Read the model definition and answer for the solid it produces. Units are mm, in the model's axes. A direction names the side the tool comes from. Coordinates: 2 decimals unless noted, no trailing zeros. Order: outer loops, then holes, each group sorted by start corner. A loop starts at its lowest first (then second) coordinate and runs counter-clockwise, first axis right, second up. Notation, with made-up numbers: (17, 84.5) - (22, 84.5) arc R19 cw to (22, 115.5) - close; hole circle Ø10 at (39, -32). An arc over 180 degrees is marked (long way). Write item = value, one per line.
from build123d import *

# Parameters (mm, degrees)
BASE_BLOCK_DEPTH             = 60
SADDLE_ARCH_DEPTH            = 60
BEARING_SEAT_CUT_FRONT_DEPTH = 10
BEARING_START                = -10
BEARING_SEAT_CUT_REAR_DEPTH  = 10
OIL_HOLE_SKETCH_R            = 8
OIL_HOLE_8_DEPTH             = 100
LOCATING_SLOTS_SKETCH_W      = 8
LOCATING_SLOTS_SKETCH_H      = 16
LOCATING_SLOTS_DEPTH         = 9


with BuildPart() as part:
    # Base Block Profile → Base Block (new body)
    with BuildSketch(Plane.XY):
        Polygon((0, 0), (53, 0), (53, 12), (70, 12), (70, 32), (44.5, 32), (44.508364197, 12), (8.257120322, 12), (8.257120322, 32), (-17, 32), (-17, 12), (0, 12), align=None)
    extrude(amount=-BASE_BLOCK_DEPTH)

    # Saddle Arch Profile → Saddle Arch (add)
    with BuildSketch(Plane.XY):
        with BuildLine():
            Line((1.378560161, 32), (8.257120322, 32))
            Line((8.257120322, 32), (8.378560161, 32))
            ThreePointArc((8.378560161, 32), (26.378560161, 50), (44.378560161, 32))
            Line((44.378560161, 32), (44.5, 32))
            Line((44.5, 32), (51.378560161, 32))
            ThreePointArc((51.378560161, 32), (26.378560161, 57), (1.378560161, 32))
        make_face()
    extrude(amount=-SADDLE_ARCH_DEPTH)

    # Bearing Seat Front Profile → Bearing Seat Cut Front (cut)
    with BuildSketch(Plane.XY):
        with BuildLine():
            Line((1.378560161, 32), (8.257120322, 32))
            Line((8.257120322, 32), (8.378560161, 32))
            ThreePointArc((8.378560161, 32), (26.378560161, 50), (44.378560161, 32))
            Line((44.378560161, 32), (44.5, 32))
            Line((44.5, 32), (51.378560161, 32))
            ThreePointArc((51.378560161, 32), (26.378560161, 57), (1.378560161, 32))
        make_face()
    extrude(amount=-BEARING_SEAT_CUT_FRONT_DEPTH, mode=Mode.SUBTRACT)

    # Bearing Seat Rear Profile → Bearing Seat Cut Rear (cut)
    with BuildSketch(Plane(origin=(0, 0, -60), x_dir=(-1, 0, 0), z_dir=(0, 0, -1)).offset(BEARING_START)):
        with BuildLine():
            Line((-51.378560161, 32), (-44.378560161, 32))
            ThreePointArc((-44.378560161, 32), (-26.378560161, 50), (-8.378560161, 32))
            Line((-8.378560161, 32), (-1.378560161, 32))
            ThreePointArc((-1.378560161, 32), (-26.378560161, 57), (-51.378560161, 32))
        make_face()
    extrude(amount=BEARING_SEAT_CUT_REAR_DEPTH, mode=Mode.SUBTRACT)

    # Oil Hole Sketch → Oil Hole Ø8 (cut)
    with BuildSketch(Plane.XZ):
        with Locations(Location((26.5, -30, 0), (0, 0, 270))):
            Circle(OIL_HOLE_SKETCH_R)
    extrude(amount=-OIL_HOLE_8_DEPTH, mode=Mode.SUBTRACT)

    # Locating Slots Sketch → Locating Slots (cut)
    with BuildSketch(Plane(origin=(0, 32, 0), x_dir=(1, 0, 0), z_dir=(0, 1, 0))):
        with Locations((-13, 30)):
            Rectangle(LOCATING_SLOTS_SKETCH_W, LOCATING_SLOTS_SKETCH_H)
        Polygon((70, 30), (70, 38), (62, 38), (62, 22), (70, 22), align=None)
    extrude(amount=-LOCATING_SLOTS_DEPTH, mode=Mode.SUBTRACT)


solid = part.part
1) For faces 1 (the face through (62, 28, -30)), 2 (the face through (-9, 12, -30)), 3 (the face through (8.257, 22, -30)), 4 (the face through (-13, 28, -38)), determine the directions among +Z, -Z, +X, -X, +Y, -Y from which every point of the face is accessible in a straight line to the end or side of a thin tool.
Returned:
face_1 = +X, +Y
face_2 = +Z, -Z, -X, -Y
face_3 = +Z, -Z
face_4 = -X, +Y
2) The part is cut by section D-D (x = 43). Determine the outline of the cut face in (y, z).
Returned:
outline = (0, -60) - (12, -60) - (12, 0) - (0, 0) - close; (38.91, -50) - (50.67, -50) - (50.67, -10) - (38.91, -10) - close
3) Flat-ended cylindrical pins translate along their axes: pin 1 Ø2 at (x, z) = (48, -39) entering from -Y; pin 2 Ø10 at (x, y) = (42, 40) entering from -Z; pin 3 Ø7.5 at (x, y) = (15, 43) entering from +Z; pin 4 Ø1.5 at (y, z) = (27, -34) entering from +X. Find the tip coordinate at first contact, or state that the pin passes through.
Returned:
pin_1 = 0
pin_2 = -50
pin_3 = -10
pin_4 = 62
4) The part is cut by section B-B (x = 26.5). Determine the outline of the cut face in (y, z).
Returned:
outline = (0, -60) - (12, -60) - (12, -38) - (0, -38) - close; (0, -22) - (12, -22) - (12, 0) - (0, 0) - close; (50, -50) - (57, -50) - (57, -38) - (50, -38) - close; (50, -22) - (57, -22) - (57, -10) - (50, -10) - close
5) The part is cut by section C-C (z = -4.5). Determine the outline of the cut face in (x, y).
Returned:
outline = (-17, 12) - (0, 12) - (0, 0) - (53, 0) - (53, 12) - (70, 12) - (70, 32) - (44.5, 32) - (44.51, 12) - (8.26, 12) - (8.26, 32) - (-17, 32) - close
6) Straight lines are drawn through the part: line 1 along X through (y, z) = (16, -42.5); line 2 along Z through (x, y) = (65, 25.5); line 3 along Z through (x, y) = (26, 51). For each, find the intervals that lie inside material, in ascending order. Write a range as from..to.
Returned:
line_1 = -17..8.26, 44.51..70
line_2 = -60..-38, -22..0
line_3 = -50..-37.98, -22.02..-10
7) The part is cut by section A-A (z = -41.5). Determine the outline of the cut face in (x, y).
Returned:
outline = (-17, 12) - (0, 12) - (0, 0) - (53, 0) - (53, 12) - (70, 12) - (70, 32) - (51.38, 32) arc R25 ccw to (1.38, 32) - (-17, 32) - close; hole (8.26, 12) - (44.51, 12) - (44.5, 32) - (44.38, 32) arc R18 ccw to (8.38, 32) - (8.26, 32) - close
8) Determine the mould class of faces 5 (the face through (26, 9, -60)), 6 (the face through (53, 6, -30)), 7 (the face through (66, 28, -22)), 8 (the face through (26, 50.2, -10)) for opening direction Z: pulls with the +Z half, pulls with the -Z half, needs draft (parallel to the pull), parting line crosses it, or undercut.
Returned:
face_5 = pulls with the -Z half
face_6 = needs draft
face_7 = undercut
face_8 = pulls with the +Z half
